Here's how the part is built. I have some questions about the finished solid (model axes, mm). A direction names the side the tool comes from. Coordinates: 2 decimals unless noted, no trailing zeros. Write each loop counter-clockwise with the first axis right and the second up, starting at its lowest first coordinate (ties: lowest second). Pieces come first, ordered by that corner, then holes. Notation, with made-up numbers: M -0.5,67 L 9.5,67 A19 ccw 9.5,80 Z; hole C 4,6.25 d6. An arc over 180 degrees is marked long. Use one line per item in the form item = value. Start each with the question number.
1. On a 3-axis mill with a long thin cutter (end or side, diameter ignored), from which of +Z, -Z, +X, -X, +Y, -Y can I reach the whole of each face in a straight line? I mean faces 4 (the face through (26.35, -7.04, 89.76)), 5 (the face through (7, -114.4, 371.7)), 6 (the face through (10, -73, 192)), 7 (the face through (13, -8, 100)). Say none if no direction works.
2. I want a section at C-C, the plane z = 269. List the corners of the cut face in (x, y) for me.
3. Please list where these lines run through material, in increasing order: line 1 along Y through (x, z) = (6.85, 375); line 2 along X through (y, z) = (-35.5, 353); line 3 along Z through (x, y) = (8, -110). Write a range as [from, to].
4. I want a section at A-A, the plane x = 30. List the corners of the cut face in (y, z) for me, plus the area to 3 significant figures.
5. Thinking about a two-plate mould opening in Z: for faces 1 (the face through (5.07, -35.703, 383.986)), 2 (the face through (4, -4.2, 49.3)), 3 (the face through (30, -4, 85)), which applies, released by +Z, released by -Z, zero draft, split by the parting line, or undercut?
6. I'm going to push flat-ended pins straight in: pin 1 Ø3.5 at (y, z) = (-110.5, 376.5) entering from +X; pin 2 Ø2 at (y, z) = (-38.5, 138) entering from -X; pin 3 Ø15.5 at (x, z) = (30, 48) entering from -Y; pin 4 Ø22 at (x, y) = (7.5, -7.5) entering from +Z. Where does each tip first touch, or does it pass through?
7. I want a section at B-B, the plane z = 15. List the corners of the cut face in (x, y) for me, plus the area to 3 significant figures.
from build123d import *

# Parameters (mm, degrees)
EXTRUDE_THIN1_DEPTH = 100
SKETCH2_W           = 10
SKETCH2_H           = 100
BOSS_EXTRUDE1_DEPTH = 290
FILLET1_R           = 10
FILLET3_R           = 20
FILLET4_R           = 60
SKETCH3_R           = 6
CUT_EXTRUDE1_DEPTH  = 6
LPATTERN1_COUNT     = 2
LPATTERN1_PITCH     = 70
SKETCH4_R           = 5.5
CUT_EXTRUDE2_DEPTH  = 6
LPATTERN2_COUNT     = 2
LPATTERN2_PITCH     = 60


with BuildPart() as part:
    # Sketch1 → Extrude-Thin1 (new body)
    with BuildSketch(Plane.XY):
        with BuildLine():
            Line((0, -130), (0, -14))
            ThreePointArc((0, -14), (4.100505063, -4.100505063), (14, 0))
            Line((14, 0), (45, 0))
            Line((45, 0), (45, -10))
            Line((45, -10), (14, -10))
            ThreePointArc((14, -10), (11.171572875, -11.171572875), (10, -14))
            Line((10, -14), (10, -130))
            Line((10, -130), (0, -130))
        make_face()
    extrude(amount=EXTRUDE_THIN1_DEPTH)

    # Sketch2 → Boss-Extrude1 (add)
    with BuildSketch(Plane.XY.offset(100)):
        with Locations((5, -80)):
            Rectangle(SKETCH2_W, SKETCH2_H)
    extrude(amount=BOSS_EXTRUDE1_DEPTH)

    # Fillet1
    fillet1_edges = [part.edges().sort_by_distance(p)[0] for p in [
        (5, -30, 100),
    ]]
    fillet(fillet1_edges, radius=FILLET1_R)

    # Fillet3
    fillet3_edges = [part.edges().sort_by_distance(p)[0] for p in [
        (5, -30, 390),
        (5, -130, 390),
        (45, -5, 0),
        (45, -5, 100),
    ]]
    fillet(fillet3_edges, radius=FILLET3_R)

    # Fillet4
    fillet4_edges = [part.edges().sort_by_distance(p)[0] for p in [
        (5, -130, 0),
    ]]
    fillet(fillet4_edges, radius=FILLET4_R)

    # Sketch3 → Cut-Extrude1 (cut)
    with BuildSketch(Plane.XZ.offset(10)):
        with Locations(Location((30, 15, 0), (0, 0, 270))):
            Circle(SKETCH3_R)
    cut_extrude1 = extrude(amount=-CUT_EXTRUDE1_DEPTH, mode=Mode.SUBTRACT)

    # LPattern1: Cut-Extrude1 ×2
    with Locations(*[(0, 0, i * LPATTERN1_PITCH) for i in range(1, LPATTERN1_COUNT)]):
        add(cut_extrude1, mode=Mode.SUBTRACT)

    # Sketch4 → Cut-Extrude2 (cut)
    with BuildSketch(Plane(origin=(10, 0, 0), x_dir=(0, 0, -1), z_dir=(1, 0, 0))):
        with Locations(Location((-375, -50, 0), (0, 0, 90))):
            Circle(SKETCH4_R)
    cut_extrude2 = extrude(amount=-CUT_EXTRUDE2_DEPTH, mode=Mode.SUBTRACT)

    # LPattern2: Cut-Extrude2 ×2
    with Locations(*[(0, -i * LPATTERN2_PITCH, 0) for i in range(1, LPATTERN2_COUNT)]):
        add(cut_extrude2, mode=Mode.SUBTRACT)


solid = part.part
Answer list:
q1.face_4 = -Y
q1.face_5 = +X
q1.face_6 = +Z, -Z, +X, -Y
q1.face_7 = +Z, +X, -X, +Y
q2.outline = M 0,-130 L 10,-130 L 10,-30 L 0,-30 Z
q3.line_1 = [-129.36, -115.5], [-104.5, -55.5], [-44.5, -30.64]
q3.line_2 = [0, 10]
q3.line_3 = [15.28, 369.5], [380.5, 390]
q4.outline = M -10,0.64 L 0,0.64 L 0,99.36 L -10,99.36 L -10,91 L -4,91 L -4,79 L -10,79 L -10,21 L -4,21 L -4,9 L -10,9 Z
q4.area = 843 mm²
q5.face_1 = released by +Z
q5.face_2 = zero draft
q5.face_3 = undercut
q6.pin_1 = 4
q6.pin_2 = 0
q6.pin_3 = -10
q6.pin_4 = 100
q7.outline = M 0,-109.69 L 10,-109.69 L 10,-14 A4 cw 14,-10 L 24,-10 L 24,-4 L 36,-4 L 36,-10 L 44.36,-10 L 44.36,0 L 14,0 A14 ccw 0,-14 Z
q7.area = 1,330 mm²
